Answer from the drawing. Dimensions are ordinates in mm from the lowest x, y and z of the part. A direction names the side the tool comes from. Give positions to 0.01 mm unless a question says otherwise; leave off trailing zeros. Write each loop counter-clockwise with the first axis right and the second up, starting at its lowest first coordinate (ties: lowest second). Pieces come first, ordered by that corner, then holes. Notation, with made-up numbers: (26, 16.25) -> (58, 16.25) arc R35 ccw to (58, 52.25) -> close; hole circle Ø6 at (2.25, -29.5). An arc over 180 degrees is marked (long way). Put each result on its own line as item: value. Start each with the question number.
1) Flat-ended cylindrical pins translate along their axes: pin 1 Ø7 at (x, y) = (23.5, 7.5) entering from +Z; pin 2 Ø6 at (x, y) = (26.5, 9) entering from +Z. Find the tip coordinate at first contact, or state that the pin passes through.
2) A cutting plane is placed at B-B (y = 7.5). Write down the section's boundary in (x, z).
3) A cutting plane is placed at D-D (y = 3.5). Write down the section's boundary in (x, z), then the cut area to 3 significant figures.
4) For a pull along X with two mould halves and no side action, classify the marked faces 3, 4, 5 and 6 as released by +X, released by -X, zero draft, split by the parting line, or undercut.
5) For the marked faces 1 and 2, determine the directions among +Z, -Z, +X, -X, +Y, -Y from which every point of the face is accessible in a straight line to the end or side of a thin tool.
6) Find the intervals of material crossed by line 1 along Y through (x, z) = (23.5, 5.55); line 2 along X through (y, z) = (8.5, 5.25); line 3 along Y through (x, z) = (23.5, 3.35), in increasing order. Write a range as from..to.
7) A cutting plane is placed at A-A (x = 8.5). Write down the section's boundary in (y, z).
8) A cutting plane is placed at C-C (z = 3.75). Write down the section's boundary in (x, y).
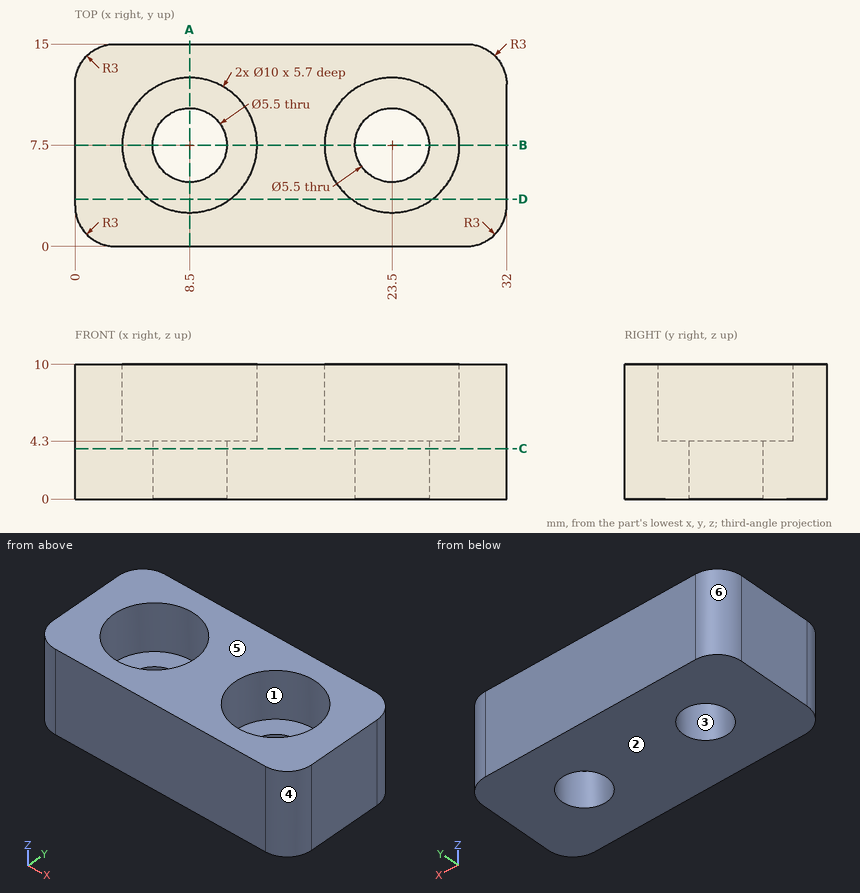
Reply:
1. pin 1: stops at z = 4.3
1. pin 2: stops at z = 10
2. outline: (0, 0) -> (5.75, 0) -> (5.75, 4.3) -> (3.5, 4.3) -> (3.5, 10) -> (0, 10) -> close; (11.25, 0) -> (20.75, 0) -> (20.75, 4.3) -> (18.5, 4.3) -> (18.5, 10) -> (13.5, 10) -> (13.5, 4.3) -> (11.25, 4.3) -> close; (26.25, 0) -> (32, 0) -> (32, 10) -> (28.5, 10) -> (28.5, 4.3) -> (26.25, 4.3) -> close
3. outline: (0, 0) -> (32, 0) -> (32, 10) -> (26.5, 10) -> (26.5, 4.3) -> (20.5, 4.3) -> (20.5, 10) -> (11.5, 10) -> (11.5, 4.3) -> (5.5, 4.3) -> (5.5, 10) -> (0, 10) -> close
3. area: 252 mm2
4. face 3: undercut
4. face 4: released by +X
4. face 5: zero draft
4. face 6: released by -X
5. face 1: +Z
5. face 2: -Z, +X, -X, +Y, -Y
6. line 1: y = 0..2.5, 12.5..15
6. line 2: x = 0..3.6, 13.4..18.6, 28.4..32
6. line 3: y = 0..4.75, 10.25..15
7. outline: (0, 0) -> (4.75, 0) -> (4.75, 4.3) -> (2.5, 4.3) -> (2.5, 10) -> (0, 10) -> close; (10.25, 0) -> (15, 0) -> (15, 10) -> (12.5, 10) -> (12.5, 4.3) -> (10.25, 4.3) -> close
8. outline: (0, 3) arc R3 ccw to (3, 0) -> (29, 0) arc R3 ccw to (32, 3) -> (32, 12) arc R3 ccw to (29, 15) -> (3, 15) arc R3 ccw to (0, 12) -> close; hole circle Ø5.5 at (8.5, 7.5); hole circle Ø5.5 at (23.5, 7.5)
